```python
from build123d import *

# Parameters (mm, degrees)
EXTRUDE_THIN1_DEPTH   = 25
SKETCH2_W             = 28.5
SKETCH2_H             = 30
BOSS_EXTRUDE1_DEPTH   = 10
SKETCH5_W             = 2
SKETCH5_H             = 22
CUT_EXTRUDE1_DEPTH    = 64.735782728
M3_TAPPED_HOLE2_D     = 2.5
SKETCH8_W             = 85.55195354
SKETCH8_H             = 65.589831047
CUT_EXTRUDE2_DEPTH    = 10
M5_TAPPED_HOLE1_D     = 4.2
M5_TAPPED_HOLE1_DEPTH = 12.4
M5_TAPPED_HOLE1_TIP   = 1.2618073
SKETCH14_W            = 4.8
SKETCH14_H            = 3
BOSS_EXTRUDE2_DEPTH   = 0.8
M3_TAPPED_HOLE1_D     = 2.5


with BuildPart() as part:
    # Sketch1 → Extrude-Thin1 (new body)
    with BuildSketch(Plane.XY):
        Polygon((-15, 0), (0, 0), (0, 45), (10, 45), (10, -10), (-15, -10), align=None)
    extrude(amount=EXTRUDE_THIN1_DEPTH)

    # Sketch2 → Boss-Extrude1 (add)
    with BuildSketch(Plane.ZY):
        with Locations((-14.25, 30)):
            Rectangle(SKETCH2_W, SKETCH2_H)
    extrude(amount=-BOSS_EXTRUDE1_DEPTH)

    # Sketch5 → Cut-Extrude1 (cut, through all)
    with BuildSketch(Plane(origin=(0, 45, 0), x_dir=(1, 0, 0), z_dir=(0, 1, 0))):
        with Locations((1, 17.5)):
            Rectangle(SKETCH5_W, SKETCH5_H)
    extrude(amount=-CUT_EXTRUDE1_DEPTH, mode=Mode.SUBTRACT)

    # M3 Tapped Hole2 (through all)
    with Locations(Plane(origin=(10, 0, 0), x_dir=(0, 0, -1), z_dir=(1, 0, 0))):
        with Locations((13.5, 36.5), (23.5, 36.5)):
            Hole(M3_TAPPED_HOLE2_D / 2)

    # Sketch8 → Cut-Extrude2 (cut)
    with BuildSketch(Plane.XZ.offset(10)):
        with Locations((-7.814591053, 5.120081117)):
            Rectangle(SKETCH8_W, SKETCH8_H)
    extrude(amount=-CUT_EXTRUDE2_DEPTH, mode=Mode.SUBTRACT)

    # M5 Tapped Hole1
    with Locations(Plane(origin=(0, 0, 0), x_dir=(-1, 0, 0), z_dir=(0, -1, 0))):
        with Locations((-5, -5.5), (-5, -19.5)):
            Hole(M5_TAPPED_HOLE1_D / 2, depth=M5_TAPPED_HOLE1_DEPTH)
            with Locations((0, 0, -(M5_TAPPED_HOLE1_DEPTH + M5_TAPPED_HOLE1_TIP / 2))):  # 118° drill point
                Cone(0, M5_TAPPED_HOLE1_D / 2, M5_TAPPED_HOLE1_TIP, mode=Mode.SUBTRACT)

    # Sketch14 → Boss-Extrude2 (add)
    with BuildSketch(Plane(origin=(10, 0, 0), x_dir=(0, 0, -1), z_dir=(1, 0, 0))):
        with Locations((24.3, 19)):
            Rectangle(SKETCH14_W, SKETCH14_H)
    extrude(amount=BOSS_EXTRUDE2_DEPTH)

    # M3 Tapped Hole1 (through all)
    with Locations(Plane.ZY):
        with Locations((-24.3, 19)):
            Hole(M3_TAPPED_HOLE1_D / 2)


solid = part.part
```
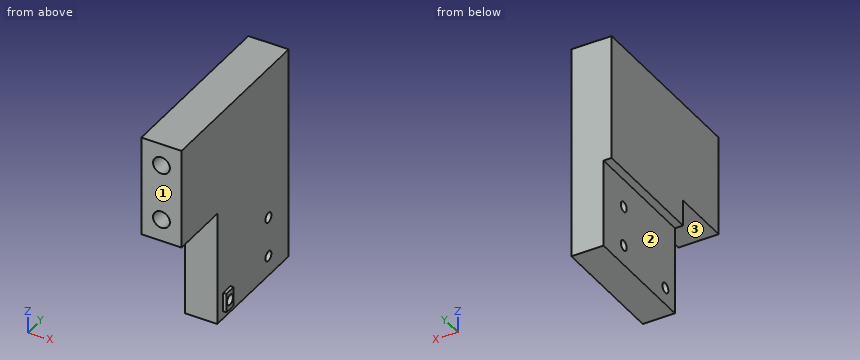
CAD build for the part. Positions are in the model's coordinates, mm. Face numbers are marked on the shaded views. A direction names the side the tool comes from. Round coordinates to 2 decimals unless told otherwise and drop trailing zeros. Order: outer loops, then holes, each group sorted by start corner. A loop starts at its lowest first (then second) coordinate and runs counter-clockwise, first axis right, second up. Notation, with made-up numbers: (-38, -25) - (14, -25) arc R25 ccw to (14, -3) - close; hole circle Ø9 at (9, 13). An arc over 180 degrees is marked (long way). Answer as CSV lines item,"result". Start each with the question number.
1. Drill centre lines: L1, parallel to Z at x = 5, y = 8; L2, parallel to Y at x = 5.25, z = -13.5; L3, parallel to Z at x = 4.25, y = 2.5. Where is each one in solid material? Low to high. Write a range as [from, to].
2. Pin check, flat tips, straight feed: pin 1 (4 mm diameter, centred on x = 5, z = 19.5, fed in from -Y); pin 2 (0.6 mm diameter, centred on x = 10.5, z = -24, fed in from -Y); pin 3 (6 mm diameter, centred on x = 9, y = 8.5, fed in from -Z). Stop position of each tip, or through.
3. Saw through at D-D, the plane y = 19. Write the cut outline in (x, z).
4. Tool access for the marked faces 1, 2 and 3: list every direction of +Z, -Z, +X, -X, +Y, -Y with a clear straight run to the whole face (end or side of a thin tool).
5. Saw through at C-C, the plane x = 8.25. Write the cut outline in (y, z).
6. Saw through at A-A, the plane y = 36.5. Write the cut outline in (x, z).
7. Saw through at B-B, the plane y = 5.5. Write the cut outline in (x, z).
Model answer:
1,L1,"z = [0, 3.4], [7.6, 17.4], [21.6, 25]"
1,L2,"y = [15, 35.25], [37.75, 45]"
1,L3,"z = [0, 3.54], [7.46, 17.54], [21.46, 25]"
2,pin 1,"stops at y = 12.46"
2,pin 2,"stops at y = 17.5"
2,pin 3,"stops at z = 0"
3,outline,"(0, -6.5) - (2, -6.5) - (2, -23.05) - (10.8, -23.05) - (10.8, -21.9) - (10, -21.9) - (10, 25) - (0, 25) - close; (2, -28.5) - (10, -28.5) - (10, -26.7) - (10.8, -26.7) - (10.8, -25.55) - (2, -25.55) - close"
4,face 1,"+Z, -Z, +X, -X, -Y"
4,face 2,"-Z, -X, +Y, -Y"
4,face 3,"-Z, +X, -X, -Y"
5,outline,"(0, 0) - (15, 0) - (15, -28.5) - (45, -28.5) - (45, 25) - (0, 25) - close; hole circle Ø2.5 at (19, -24.3); hole circle Ø2.5 at (36.5, -23.5); hole circle Ø2.5 at (36.5, -13.5)"
6,outline,"(0, -6.5) - (2, -6.5) - (2, -12.25) - (10, -12.25) - (10, 25) - (0, 25) - close; (2, -28.5) - (10, -28.5) - (10, -24.75) - (2, -24.75) - close; (2, -22.25) - (10, -22.25) - (10, -14.75) - (2, -14.75) - close"
7,outline,"(0, 0) - (10, 0) - (10, 25) - (0, 25) - close; hole circle Ø4.2 at (5, 5.5); hole circle Ø4.2 at (5, 19.5)"
